```python
from build123d import *

# Parameters (mm, degrees)
BASE_PLATE_SKETCH_W         = 290
BASE_PLATE_SKETCH_H         = 30
BASE_PLATE_DEPTH            = 50
BEARING_BOSS_SKETCH_R       = 50
BEARING_BOSS_SKETCH_R_2     = 30
BEARING_BOSS_DEPTH          = 56
BASE_MOUNTING_CUT_SKETCH_R  = 12.5
BASE_MOUNTING_CUT_DEPTH     = 56
SUPPORT_LUG_SKETCH_W        = 194
SUPPORT_LUG_SKETCH_H        = 25
SUPPORT_LUG_DEPTH           = 130
LUG_PIN_HOLE_SKETCH_R       = 12.5
LUG_PIN_HOLE_25_DEPTH       = 65
LUG_PROFILE_CUT_DEPTH       = 130
HOUSING_CLEARANCE_CUT_DEPTH = 110
BEARING_START               = -120
BEARING_BORE_SKETCH_R       = 30
BEARING_BORE_60_DEPTH       = 120
RIB_1_DEPTH                 = 25
RIB_2_DEPTH                 = 25
RIB_3_DEPTH                 = 25
RIB_4_DEPTH                 = 25


with BuildPart() as part:
    # Base Plate Sketch → Base Plate (new, symmetric)
    with BuildSketch(Plane.XY):
        with Locations((-35, 15)):
            Rectangle(BASE_PLATE_SKETCH_W, BASE_PLATE_SKETCH_H)
    extrude(amount=BASE_PLATE_DEPTH, both=True)

    # Base Mounting Cut Sketch → Base Mounting Cut (cut, symmetric)
    with BuildSketch(Plane(origin=(0, 0, 0), x_dir=(1, 0, 0), z_dir=(0, 1, 0))):
        with Locations(Location((-144, 0, 0), (0, 0, 180))):
            Circle(BASE_MOUNTING_CUT_SKETCH_R)
        with Locations(Location((74, 0, 0), (0, 0, 180))):
            Circle(BASE_MOUNTING_CUT_SKETCH_R)
    extrude(amount=BASE_MOUNTING_CUT_DEPTH, both=True, mode=Mode.SUBTRACT)



with BuildPart() as body_2:
    # Bearing Boss Sketch → Bearing Boss (new, symmetric)
    with BuildSketch(Plane.XY):
        with Locations((0, 100)):
            Circle(BEARING_BOSS_SKETCH_R)
        with Locations((0, 100)):
            Circle(BEARING_BOSS_SKETCH_R_2, mode=Mode.SUBTRACT)
    extrude(amount=BEARING_BOSS_DEPTH, both=True)


with BuildPart() as part_1:
    add(part.part)

    add(body_2.part)  # Support Lug merges body 2
    # Support Lug Sketch → Support Lug (add)
    with BuildSketch(Plane(origin=(0, 0, 0), x_dir=(1, 0, 0), z_dir=(0, 1, 0))):
        with Locations((-23, -37.5)):
            Rectangle(SUPPORT_LUG_SKETCH_W, SUPPORT_LUG_SKETCH_H)
    support_lug = extrude(amount=SUPPORT_LUG_DEPTH)

    # Support Lug Mirror: Support Lug across plane
    add(support_lug.mirror(Plane.XY))

    # Lug Pin Hole Sketch → Lug Pin Hole Ø25 (cut, symmetric)
    with BuildSketch(Plane.XY):
        with Locations((-90, 100)):
            Circle(LUG_PIN_HOLE_SKETCH_R)
    extrude(amount=LUG_PIN_HOLE_25_DEPTH, both=True, mode=Mode.SUBTRACT)

    # Lug Profile Cut Sketch → Lug Profile Cut (cut)
    with BuildSketch(Plane.XY.offset(50)):
        with BuildLine():
            Line((-120, 100), (-120, 130))
            Line((-120, 130), (-90, 130))
            ThreePointArc((-90, 130), (-111.213203436, 121.213203436), (-120, 100))
        make_face()
    extrude(amount=-LUG_PROFILE_CUT_DEPTH, mode=Mode.SUBTRACT)

    # Housing Clearance Sketch → Housing Clearance Cut (cut)
    with BuildSketch(Plane.XY.offset(50)):
        with BuildLine():
            Line((74, 130), (44, 130))
            ThreePointArc((44, 130), (65.213203436, 121.213203436), (74, 100))
            Line((74, 100), (74, 130))
        make_face()
    extrude(amount=-HOUSING_CLEARANCE_CUT_DEPTH, mode=Mode.SUBTRACT)

    # Bearing Bore Sketch → Bearing Bore Ø60 (cut)
    with BuildSketch(Plane.XY.offset(56).offset(BEARING_START)):
        with Locations((0, 100)):
            Circle(BEARING_BORE_SKETCH_R)
    extrude(amount=BEARING_BORE_60_DEPTH, mode=Mode.SUBTRACT)

    # Rib 1 Sketch → Rib 1 (add)
    with BuildSketch(Plane.XY.offset(50)):
        with BuildLine():
            Line((-127.5, 30), (-120, 30))
            Line((-120, 30), (-120, 37.5))
            ThreePointArc((-120, 37.5), (-122.196699141, 32.196699141), (-127.5, 30))
        make_face()
    extrude(amount=-RIB_1_DEPTH)

    # Rib 2 Sketch → Rib 2 (add)
    with BuildSketch(Plane.XY.offset(-25)):
        with BuildLine():
            Line((-127.5, 30), (-120, 30))
            Line((-120, 30), (-120, 37.5))
            ThreePointArc((-120, 37.5), (-122.196699141, 32.196699141), (-127.5, 30))
        make_face()
    extrude(amount=-RIB_2_DEPTH)

    # Rib 3 Sketch → Rib 3 (add)
    with BuildSketch(Plane.XY.offset(50)):
        with BuildLine():
            Line((74, 37.5), (74, 30))
            Line((74, 30), (81.5, 30))
            ThreePointArc((81.5, 30), (76.196699141, 32.196699141), (74, 37.5))
        make_face()
    extrude(amount=-RIB_3_DEPTH)

    # Rib 4 Sketch → Rib 4 (add)
    with BuildSketch(Plane.XY.offset(-25)):
        with BuildLine():
            Line((74, 30), (81.5, 30))
            ThreePointArc((81.5, 30), (76.196699141, 32.196699141), (74, 37.5))
            Line((74, 37.5), (74, 30))
        make_face()
    extrude(amount=-RIB_4_DEPTH)


solid = part_1.part
```
For this review, take the finished solid that the model builds, in its own axes (mm). A direction names the side the tool comes from. Give positions to 0.01 mm unless a question says otherwise; leave off trailing zeros. Loops run counter-clockwise (first coordinate to the right, second up) from the corner with the lowest first, then second, coordinate; pieces in that order, holes last. Notation, with made-up numbers: M -23.75,71.5 L 24.25,71.5 A13 cw 24.25,94.5 Z; hole C 64.5,55 d9. An arc over 180 degrees is marked long. One line per item, written item: value. Start each with the question number.
Q1. Add section B-B (z = 0). Give the boundary of the cut face in (x, y), and give its area (3 significant figures).
Q2. Clearance check with flat-ended pins moving along their axes: pin 1 Ø2 at (x, z) = (43, 42.5) entering from +Y; pin 2 Ø10 at (x, z) = (-110.5, 0.5) entering from +Y; pin 3 Ø10 at (x, y) = (59, 60) entering from +Z; pin 4 Ø20 at (x, z) = (-144, 0) entering from +Y. State where each tip first meets the part, or that it passes through.
Q3. Add section A-A (x = 0). Give the boundary of the cut face in (y, z), and give its area (3 significant figures).
Q4. Add section C-C (x = -144). Give the boundary of the cut face in (y, z).
Q5. Machinability: for faces 4 (the face through (-120, 68, -38)), 5 (the face through (-6.509, 149.575, 0.784)), 6 (the face through (-83.28, 110.54, 37.67)), which of the approach directions +Z, -Z, +X, -X, +Y, -Y give a long, thin tool a straight path to every point of the face, cutting with its end or side? Answer none if there is none.
Q6. For L1, parallel to Z at x = -144, y = 13; L2, parallel to Z at x = -114, y = 55; L3, parallel to Y at x = -90, z = 44, list the stretches that pass through material, from the lowest coordinate up.
Q7. Draft analysis for pull direction X (two halves, no side actions). For faces 1 (the face through (-37, 51, 50)), 2 (the face through (64.979, 121.445, 37.675)), 3 (the face through (-155.923, 14.79, 3.755)), state which applies: released by +X, released by -X, zero draft, split by the parting line, or undercut.
Q8. Add section D-D (z = 40). Give the boundary of the cut face in (x, y).
Reply:
1. outline: M -180,0 L -156.5,0 L -156.5,30 L -180,30 Z; M -131.5,0 L 61.5,0 L 61.5,30 L -131.5,30 Z; C 0,100 d100; M 86.5,0 L 110,0 L 110,30 L 86.5,30 Z; hole C 0,100 d60
1. area: 12,200 mm²
2. pin 1: y = 130
2. pin 2: y = 30
2. pin 3: z = 50
2. pin 4: through
3. outline: M 0,-50 L 50,-50 L 50,-56 L 70,-56 L 70,56 L 50,56 L 50,50 L 0,50 Z; M 130,-56 L 150,-56 L 150,56 L 130,56 Z; hole M 30,-25 L 50,-25 L 50,25 L 30,25 Z
3. area: 8,480 mm²
4. outline: M 0,-50 L 30,-50 L 30,-12.5 L 0,-12.5 Z; M 0,12.5 L 30,12.5 L 30,50 L 0,50 Z
5. face 4: +Z, -Z, -X, +Y
5. face 5: none
5. face 6: +Z, -Z
6. L1: -50 to -12.5, 12.5 to 50
6. L2: -50 to -25, 25 to 50
6. L3: 0 to 87.5, 112.5 to 130
7. face 1: zero draft
7. face 2: released by +X
7. face 3: undercut
8. outline: M -180,0 L 110,0 L 110,30 L 81.5,30 A7.5 cw 74,37.5 L 74,100 A30 ccw 44,130 L 40,130 A50 ccw -40,130 L -90,130 A30 ccw -120,100 L -120,37.5 A7.5 cw -127.5,30 L -180,30 Z; hole C -90,100 d25; hole C 0,100 d60
